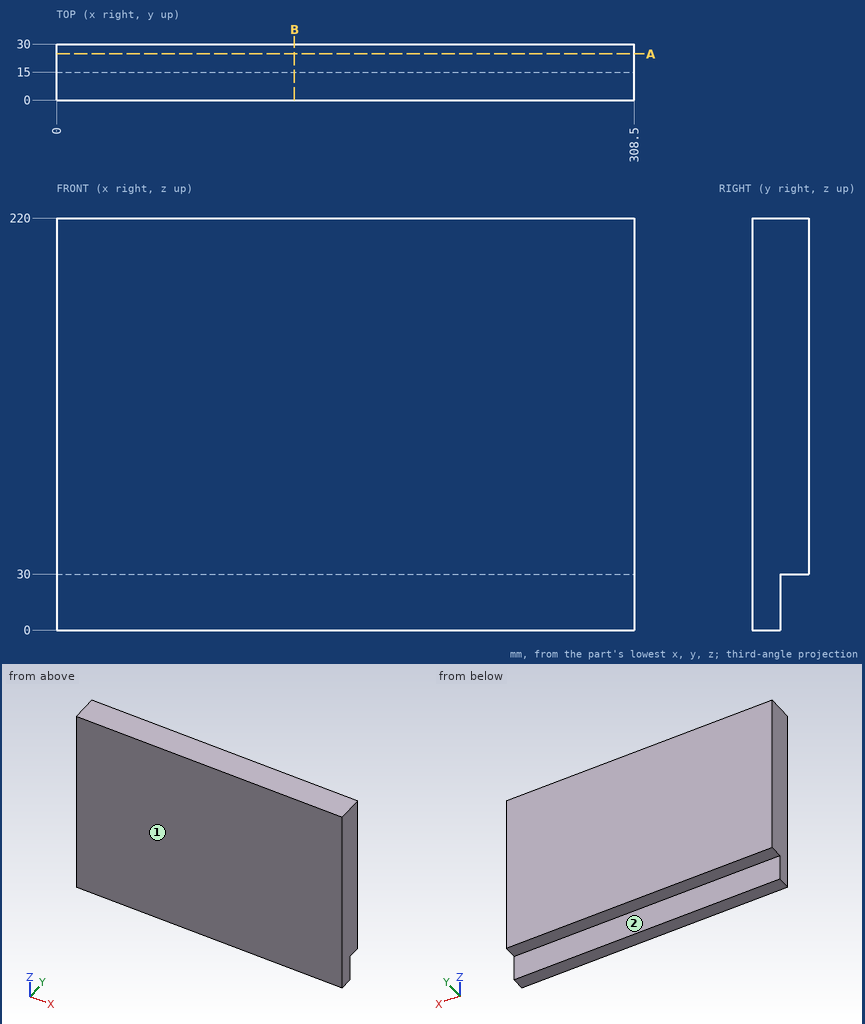
Can you work these out from the drawing? Everything is in mm from the part's minimum corner. A direction names the side the tool comes from. Give positions to 0.01 mm unless a question says otherwise; leave off trailing zeros. Loops run counter-clockwise (first coordinate to the right, second up) from the corner with the lowest first, then second, coordinate; pieces in that order, holes last. Notation, with made-up numbers: (71.25, 71.5) -> (75.25, 71.5) arc R28 ccw to (75.25, 95.5) -> close; hole circle Ø9 at (31, 55). An arc over 180 degrees is marked (long way). Write item = value, one per line.
1) For the marked faces 1 and 2, which set-ups out of +Z, -Z, +X, -X, +Y, -Y let a thin tool reach every point of the face, with its end or its side?
Check result:
face_1 = +Z, -Z, +X, -X, -Y
face_2 = -Z, +X, -X, +Y
2) I need wall thicknesses on L1, parallel to Y at x = 241.5, z = 20.5; L2, parallel to Z at x = 252, y = 25.5. Which ranges of each line are inside material? Lowest first, please. Write a range as from..to.
Check result:
L1 = 0..15
L2 = 30..220
3) Suppose I cut it at B-B on x = 127. Write out the boundary of the cut face in (y, z), then the cut area to 3 significant figures.
Check result:
outline = (0, 0) -> (15, 0) -> (15, 30) -> (30, 30) -> (30, 220) -> (0, 220) -> close
area = 6,150 mm2
4) Will these pins go through, and if not, where does the flat tip stop? pin 1 (24 mm diameter, centred on x = 99, z = 13, fed in from +Y); pin 2 (7.5 mm diameter, centred on x = 227, y = 22, fed in from -Z).
Check result:
pin_1 = 15
pin_2 = 30
5) Suppose I cut it at A-A on y = 24.75. Write out the boundary of the cut face in (x, z), then the cut area to 3 significant figures.
Check result:
outline = (0, 30) -> (308.5, 30) -> (308.5, 220) -> (0, 220) -> close
area = 58,600 mm2
